```python
from build123d import *

# Parameters (mm, degrees)
SKETCH1_R           = 3
BOSS_EXTRUDE1_DEPTH = 20.5
SKETCH2_R           = 4
BOSS_EXTRUDE2_DEPTH = 1.2
SKETCH5_R           = 3
BOSS_EXTRUDE3_DEPTH = 23.2
CHAMFER3_SIZE       = 0.5
BOSS_EXTRUDE4_START = 20.5
SKETCH6_R           = 4
BOSS_EXTRUDE4_DEPTH = 20.5
CHAMFER4_SIZE       = 0.3
SKETCH9_R           = 5
BOSS_EXTRUDE5_DEPTH = 20
CHAMFER5_SIZE       = 0.5
SKETCH10_W          = 1
SKETCH10_H          = 10
CUT_EXTRUDE2_DEPTH  = 10
CIRPATTERN2_COUNT   = 2
CIRPATTERN2_ANGLE   = 135


with BuildPart() as part:
    # Sketch1 → Boss-Extrude1 (new body)
    with BuildSketch(Plane(origin=(0, 0, 0), x_dir=(1, 0, 0), z_dir=(0, 1, 0))):
        with Locations(Location((0, 0, 0), (0, 0, 270))):
            Circle(SKETCH1_R)
    extrude(amount=BOSS_EXTRUDE1_DEPTH)

    # Sketch2 → Boss-Extrude2 (add)
    with BuildSketch(Plane(origin=(0, 20.5, 0), x_dir=(1, 0, 0), z_dir=(0, 1, 0))):
        with Locations(Location((0, 0, 0), (0, 0, 270))):
            Circle(SKETCH2_R)
    extrude(amount=BOSS_EXTRUDE2_DEPTH)

    # Sketch5 → Boss-Extrude3 (add)
    with BuildSketch(Plane(origin=(0, 21.7, 0), x_dir=(1, 0, 0), z_dir=(0, 1, 0))):
        with Locations(Location((0, 0, 0), (0, 0, 270))):
            Circle(SKETCH5_R)
    extrude(amount=BOSS_EXTRUDE3_DEPTH)

    # Chamfer3
    chamfer3_edges = [part.edges().sort_by_distance(p)[0] for p in [
        (0, 44.9, -3),
    ]]
    chamfer(chamfer3_edges, length=CHAMFER3_SIZE)

    # Sketch6 → Boss-Extrude4 (add)
    with BuildSketch(Plane.XZ.offset(-20.5).offset(BOSS_EXTRUDE4_START)):
        with Locations(Location((0, 0, 0), (0, 0, 90))):
            Circle(SKETCH6_R)
    extrude(amount=-BOSS_EXTRUDE4_DEPTH)

    # Chamfer4
    chamfer4_edges = [part.edges().sort_by_distance(p)[0] for p in [
        (0, 21.7, -4),
    ]]
    chamfer(chamfer4_edges, length=CHAMFER4_SIZE)

    # Sketch9 → Boss-Extrude5 (add)
    with BuildSketch(Plane.XZ):
        with Locations(Location((0, 0, 0), (0, 0, 270))):
            Circle(SKETCH9_R)
    extrude(amount=-BOSS_EXTRUDE5_DEPTH)

    # Chamfer5
    chamfer5_edges = [part.edges().sort_by_distance(p)[0] for p in [
        (0, 0, 5),
        (0, 20, 5),
    ]]
    chamfer(chamfer5_edges, length=CHAMFER5_SIZE)

    # Sketch10 → Cut-Extrude2 (cut, symmetric)
    with BuildSketch(Plane.XY):
        with Locations((5, 9.5)):
            Rectangle(SKETCH10_W, SKETCH10_H)
    cut_extrude2 = extrude(amount=CUT_EXTRUDE2_DEPTH, both=True, mode=Mode.SUBTRACT)

    # CirPattern2: Cut-Extrude2 ×2 about axis
    cirpattern2_axis = Axis((0, 44.9, 0), (0, -1, 0))
    for i in range(1, CIRPATTERN2_COUNT):
        add(cut_extrude2.rotate(cirpattern2_axis, i * CIRPATTERN2_ANGLE / (CIRPATTERN2_COUNT - 1)), mode=Mode.SUBTRACT)


solid = part.part
```
Build history of the part. All positions in model axes, mm. A direction names the side the tool comes from. Give positions to 0.01 mm unless a question says otherwise; leave off trailing zeros. Loops run counter-clockwise (first coordinate to the right, second up) from the corner with the lowest first, then second, coordinate; pieces in that order, holes last. Notation, with made-up numbers: (-25.75, 87) -> (30.25, 87) arc R18 cw to (30.25, 114) -> close; hole circle Ø11 at (-19.75, -13.75). An arc over 180 degrees is marked (long way). One line per question, with ' | ' between items. Start each with the question number.
1) Cut at B-B (x = 0). Give the cut face in (y, z), plus the area to 3 significant figures.
2) Pin check, flat tips, straight feed: pin 1 (3.5 mm diameter, centred on y = 10.5, z = 1, fed in from +X); pin 2 (3 mm diameter, centred on y = 13.5, z = 3, fed in from -X); pin 3 (4 mm diameter, centred on y = 40.5, z = 1.5, fed in from -X). Stop position of each tip, or through.
3) Probe L1, parallel to Y at x = -2.25, z = 2.5; L2, parallel to Y at x = 3.5, z = 2; L3, parallel to X at y = 21.5, z = -2.5. List the from-to ranges inside material, lowest first.
4) Cut at D-D (y = 39). Give the cut face in (x, z).
5) Cut at A-A (z = 0). Give the cut face in (x, y).
6) 3-axis set-ups, long thin cutter, end or side, ignore diameter. For faces 1 (the flat face through (-3.3, 14.5, 3.3)), 2 (the flat face through (4.5, 9, 0)), 3 (the flat face through (-3, 20, 3)): which of +Z, -Z, +X, -X, +Y, -Y reach the whole face in a straight line?
7) Cut at C-C (y = 10). Give the cut face in (x, z), plus the area to 3 significant figures.
8) Two-plate mould, pull along Y, no slides. Class faces 4 (the flat face through (3, 21.7, -1)), 5 (the flat face through (-3.3, 4.5, 3.3)), 6 (the flat face through (-3.204, 9.43, 3.16)), 7 (the cylindrical face through (3.905, 20.69, -0.867)): released by +Y, released by -Y, zero draft, split by the parting line, or undercut.
Return value:
1) outline: (0, -4.5) -> (0.5, -5) -> (19.5, -5) -> (20, -4.5) -> (20, -4) -> (21.4, -4) -> (21.7, -3.7) -> (21.7, -3) -> (44.4, -3) -> (44.9, -2.5) -> (44.9, 2.5) -> (44.4, 3) -> (21.7, 3) -> (21.7, 3.7) -> (21.4, 4) -> (20, 4) -> (20, 4.5) -> (19.5, 5) -> (0.5, 5) -> (0, 4.5) -> close | area: 352 mm^2
2) pin 1: x = 4.5 | pin 2: x = -4.77 | pin 3: x = -3
3) L1: 0 to 21.7 | L2: 0 to 20 | L3: -2.99 to 2.99
4) outline: circle Ø6 at (0, 0)
5) outline: (-5, 0.5) -> (-4.5, 0) -> (4.5, 0) -> (5, 0.5) -> (5, 4.5) -> (4.5, 4.5) -> (4.5, 14.5) -> (5, 14.5) -> (5, 19.5) -> (4.5, 20) -> (4, 20) -> (4, 21.4) -> (3.7, 21.7) -> (3, 21.7) -> (3, 44.4) -> (2.5, 44.9) -> (-2.5, 44.9) -> (-3, 44.4) -> (-3, 21.7) -> (-3.7, 21.7) -> (-4, 21.4) -> (-4, 20) -> (-4.5, 20) -> (-5, 19.5) -> close
6) face 1: +Z, -X | face 2: +Z, -Z, +X | face 3: +Y
7) outline: (-4.72, 1.64) arc R5 ccw to (4.5, -2.18) -> (4.5, 2.18) arc R5 ccw to (-1.64, 4.72) -> close | area: 75.6 mm^2
8) face 4: released by +Y | face 5: undercut | face 6: undercut | face 7: zero draft
